```python
from build123d import *

# Parameters (mm, degrees)
BOSS_EXTRUDE1_DEPTH     = 418
SKETCH2_W               = 20
SKETCH2_H               = 220
CUT_EXTRUDE1_DEPTH      = 25
SKETCH3_W               = 125
SKETCH3_H               = 45
CUT_EXTRUDE2_DEPTH      = 482.157978215
FILLET1_R               = 3
FILLET2_R               = 1
SKETCH5_R               = 3.5
CUT_EXTRUDE4_DEPTH      = 476.524973056
CUT_EXTRUDE5_REACH      = 483.868
SKETCH6_R               = 3.5
SKETCH8_W               = 2
SKETCH8_H               = 105
BOSS_EXTRUDE2_DEPTH     = 24
SKETCH9_W               = 2
SKETCH9_H               = 105
BOSS_EXTRUDE3_DEPTH     = 24
CUT_EXTRUDE6_DEPTH      = 30
CUT_EXTRUDE6_DEPTH_BACK = 10
SKETCH10_W              = 126
SKETCH10_H              = 50
CHAMFER1_SIZE           = 10
SKETCH11_W              = 50
SKETCH11_H              = 30
CUT_EXTRUDE7_DEPTH      = 10


with BuildPart() as part:
    # Sketch1 → Boss-Extrude1 (new body)
    with BuildSketch(Plane(origin=(0, 0, 0), x_dir=(1, 0, 0), z_dir=(0, 1, 0))):
        Polygon((0, 0), (0, 165), (148, 165), (148, 15), (170, 15), (170, 17), (150, 17), (150, 167), (-2, 167), (-2, 0), align=None)
    extrude(amount=BOSS_EXTRUDE1_DEPTH)

    # Sketch2 → Cut-Extrude1 (cut)
    with BuildSketch(Plane(origin=(0, 0, -167), x_dir=(-1, 0, 0), z_dir=(0, 0, -1))):
        with Locations((-8, 209)):
            Rectangle(SKETCH2_W, SKETCH2_H)
    extrude(amount=-CUT_EXTRUDE1_DEPTH, mode=Mode.SUBTRACT)

    # Sketch3 → Cut-Extrude2 (cut, through all)
    with BuildSketch(Plane(origin=(0, 0, -167), x_dir=(-1, 0, 0), z_dir=(0, 0, -1))):
        with Locations((-107.5, 395.5)):
            Rectangle(SKETCH3_W, SKETCH3_H)
        with Locations((-107.5, 22.5)):
            Rectangle(SKETCH3_W, SKETCH3_H)
    extrude(amount=-CUT_EXTRUDE2_DEPTH, mode=Mode.SUBTRACT)

    # Fillet1
    fillet1_edges = [part.edges().sort_by_distance(p)[0] for p in [
        (-2, 368.5, -167),
        (-2, 49.5, -167),
        (150, 209, -167),
        (148, 209, -15),
    ]]
    fillet(fillet1_edges, radius=FILLET1_R)

    # Fillet2
    fillet2_edges = [part.edges().sort_by_distance(p)[0] for p in [
        (0, 368.5, -165),
        (0, 49.5, -165),
        (150, 209, -17),
        (148, 209, -165),
    ]]
    fillet(fillet2_edges, radius=FILLET2_R)

    # Sketch5 → Cut-Extrude4 (cut, through all)
    with BuildSketch(Plane(origin=(0, 0, -17), x_dir=(-1, 0, 0), z_dir=(0, 0, -1))):
        with Locations((-160, 239)):
            Circle(SKETCH5_R)
        with Locations((-160, 179)):
            Circle(SKETCH5_R)
    extrude(amount=-CUT_EXTRUDE4_DEPTH, mode=Mode.SUBTRACT)

    # Sketch6 → Cut-Extrude5 (cut, up to next)
    with BuildSketch(Plane.ZY.offset(2), mode=Mode.PRIVATE) as cut_extrude5_sk1:
        with Locations((-7.5, 309)):
            Circle(SKETCH6_R)
    cut_extrude5_tool1 = extrude(cut_extrude5_sk1.sketch, amount=-CUT_EXTRUDE5_REACH, mode=Mode.PRIVATE) & part.part
    # Sketch6 → Cut-Extrude5 (cut, up to next)
    with BuildSketch(Plane.ZY.offset(2), mode=Mode.PRIVATE) as cut_extrude5_sk2:
        with Locations((-7.5, 209)):
            Circle(SKETCH6_R)
    cut_extrude5_tool2 = extrude(cut_extrude5_sk2.sketch, amount=-CUT_EXTRUDE5_REACH, mode=Mode.PRIVATE) & part.part
    # Sketch6 → Cut-Extrude5 (cut, up to next)
    with BuildSketch(Plane.ZY.offset(2), mode=Mode.PRIVATE) as cut_extrude5_sk3:
        with Locations((-7.5, 109)):
            Circle(SKETCH6_R)
    cut_extrude5_tool3 = extrude(cut_extrude5_sk3.sketch, amount=-CUT_EXTRUDE5_REACH, mode=Mode.PRIVATE) & part.part
    add(cut_extrude5_tool1.solids().sort_by_distance((-2, 309, -7.5))[0], mode=Mode.SUBTRACT)
    add(cut_extrude5_tool2.solids().sort_by_distance((-2, 209, -7.5))[0], mode=Mode.SUBTRACT)
    add(cut_extrude5_tool3.solids().sort_by_distance((-2, 109, -7.5))[0], mode=Mode.SUBTRACT)

    # Sketch8 → Boss-Extrude2 (add)
    with BuildSketch(Plane.XZ):
        with Locations((-1, -52.5)):
            Rectangle(SKETCH8_W, SKETCH8_H)
    extrude(amount=BOSS_EXTRUDE2_DEPTH)

    # Sketch9 → Boss-Extrude3 (add)
    with BuildSketch(Plane(origin=(0, 418, 0), x_dir=(1, 0, 0), z_dir=(0, 1, 0))):
        with Locations((-1, 52.5)):
            Rectangle(SKETCH9_W, SKETCH9_H)
    extrude(amount=BOSS_EXTRUDE3_DEPTH)

    # Sketch10 → Cut-Extrude6 (cut, two sides: drawn at the far end of the back side and taken through both)
    with BuildSketch(Plane(origin=(150, 0, 0), x_dir=(0, 0, -1), z_dir=(1, 0, 0)).offset(-CUT_EXTRUDE6_DEPTH_BACK)):
        with Locations((78, 348)):
            Rectangle(SKETCH10_W, SKETCH10_H)
        with Locations((78, 70)):
            Rectangle(SKETCH10_W, SKETCH10_H)
    extrude(amount=CUT_EXTRUDE6_DEPTH + CUT_EXTRUDE6_DEPTH_BACK, mode=Mode.SUBTRACT)

    # Chamfer1
    chamfer1_edges = [part.edges().sort_by_distance(p)[0] for p in [
        (149, 373, -141),
        (149, 45, -141),
    ]]
    chamfer(chamfer1_edges, length=CHAMFER1_SIZE)

    # Sketch11 → Cut-Extrude7 (cut)
    with BuildSketch(Plane(origin=(150, 0, 0), x_dir=(0, 0, -1), z_dir=(1, 0, 0))):
        with Locations((90, 110)):
            Rectangle(SKETCH11_W, SKETCH11_H)
        with Locations((90, 308)):
            Rectangle(SKETCH11_W, SKETCH11_H)
    extrude(amount=-CUT_EXTRUDE7_DEPTH, mode=Mode.SUBTRACT)


solid = part.part
```
Here's how the part is built. I have some questions about the finished solid (model axes, mm). A direction names the side the tool comes from. Coordinates: 2 decimals unless noted, no trailing zeros. Order: outer loops, then holes, each group sorted by start corner. A loop starts at its lowest first (then second) coordinate and runs counter-clockwise, first axis right, second up.
Item 1: If we section it at C-C, the plane y = 403.5: List the corners of the cut face in (x, z) for me.
Response values:
outline: (-2, -164) arc R3 ccw to (1, -167) - (45, -167) - (45, -165) - (1, -165) arc R1 cw to (0, -164) - (0, 0) - (-2, 0) - close
Item 2: I'm going to push flat-ended pins straight in: pin 1 Ø0.6 at (x, z) = (149, -134) entering from +Y; pin 2 Ø0.6 at (x, z) = (148.5, -123.5) entering from -Y; pin 3 Ø1.6 at (x, y) = (-1, -8) entering from -Z. Where does each tip first touch, or does it pass through?
Response values:
pin 1: stops at y = 323
pin 2: stops at y = 95
pin 3: stops at z = -105
Item 3: Which directions (+Z, -Z, +X, -X, +Y, -Y) give clear straight access to the entire face, cutting with the end or side of a thin tool? Please do faces 1 (the face through (0, 206, -81)), 2 (the face through (149, 50, -146)), 3 (the face through (109, 373, -166)).
Response values:
face 1: +Z, +Y, -Y
face 2: +Z, +X, -Y
face 3: +Z, -Z, +X, +Y
Item 4: If we section it at D-D, the plane x = 61: List the corners of the cut face in (y, z) for me, then the cut area to 3 significant figures.
Response values:
outline: (45, -167) - (373, -167) - (373, -165) - (45, -165) - close
area: 656 mm2
Item 5: If we section it at B-B, the plane y = 191.5: List the corners of the cut face in (x, z) for me, then the cut area to 3 significant figures.
Response values:
outline: (-2, -142) - (0, -142) - (0, 0) - (-2, 0) - close; (18, -167) - (147, -167) arc R3 ccw to (150, -164) - (150, -18) arc R1 cw to (151, -17) - (170, -17) - (170, -15) - (151, -15) arc R3 ccw to (148, -18) - (148, -164) arc R1 cw to (147, -165) - (18, -165) - close
area: 885 mm2
Item 6: If we section it at A-A, the plane z = -51.5: List the corners of the cut face in (x, y) for me.
Response values:
outline: (-2, -24) - (0, -24) - (0, 442) - (-2, 442) - close; (148, 95) - (150, 95) - (150, 323) - (148, 323) - close
Item 7: I need wall thicknesses on probe 1 along Y at (x, z) = (-0.8, -7.5); probe 2 along X at (y, z) = (281.5, -66); probe 3 along X at (y, z) = (179, -16). Which ranges of each line are inside material? Lowest first, please.
Response values:
probe 1: y = -24 to 105.5, 112.5 to 205.5, 212.5 to 305.5, 312.5 to 442
probe 2: x = -2 to 0, 148 to 150
probe 3: x = -2 to 0, 148.76 to 156.5, 163.5 to 170
